Geometry check sheet. Reference: the model listing, model coordinates, mm. A direction names the side the tool comes from. Coordinates: 2 decimals unless noted, no trailing zeros. Write each loop counter-clockwise with the first axis right and the second up, starting at its lowest first coordinate (ties: lowest second). Pieces come first, ordered by that corner, then holes. Notation, with made-up numbers: M 53.5,47.25 L 94.5,47.25 A14 ccw 94.5,70.25 Z; hole C 22.25,20.5 d3. An arc over 180 degrees is marked long. Write each question's results on one line, items separated by ' | '.
```python
from build123d import *

# Parameters (mm, degrees)
BOSS_EXTRUDE1_DEPTH                                = 75
HOLE_SIZE_SOCKET_HEAD_CAP_SCREW_TYPE_1_D           = 4.5
HOLE_SIZE_SOCKET_HEAD_CAP_SCREW_TYPE_1_CBORE_D     = 8
HOLE_SIZE_SOCKET_HEAD_CAP_SCREW_TYPE_1_CBORE_DEPTH = 4.6
M5_TAPPED_HOLE1_D                                  = 4.2
M5_TAPPED_HOLE1_DEPTH                              = 12.4
M5_TAPPED_HOLE1_TIP                                = 1.2618073
M5_TAPPED_HOLE2_D                                  = 4.2
M5_TAPPED_HOLE2_DEPTH                              = 12.4
M5_TAPPED_HOLE2_TIP                                = 1.2618073
CHAMFER1_SIZE                                      = 1
DOWEL_HOLE1_D                                      = 5
DOWEL_HOLE1_DEPTH                                  = 7.5
DOWEL_HOLE1_TIP                                    = 1.502151548


with BuildPart() as part:
    # Sketch1 → Boss-Extrude1 (new, symmetric)
    with BuildSketch(Plane.XY):
        Polygon((0, 0), (0, 22), (-38, 22), (-38, 2), (-2, 2), (-2, 0), align=None)
    extrude(amount=BOSS_EXTRUDE1_DEPTH, both=True)

    # Hole size (socket head cap screw type)1 (through all)
    with Locations(Plane(origin=(0, 22, 0), x_dir=(1, 0, 0), z_dir=(0, 1, 0))):
        with Locations((-32, -68.3), (-32, 68.3), (-6, 42.3), (-32, 42.3), (-6, 68.3), (-6, -68.3), (-6, -42.3), (-32, -42.3)):
            CounterBoreHole(HOLE_SIZE_SOCKET_HEAD_CAP_SCREW_TYPE_1_D / 2, HOLE_SIZE_SOCKET_HEAD_CAP_SCREW_TYPE_1_CBORE_D / 2, HOLE_SIZE_SOCKET_HEAD_CAP_SCREW_TYPE_1_CBORE_DEPTH)

    # M5 Tapped Hole1
    with Locations(Plane(origin=(0, 0, 0), x_dir=(0, 0, -1), z_dir=(1, 0, 0))):
        with Locations((0, 12), (-25, 12), (25, 12)):
            Hole(M5_TAPPED_HOLE1_D / 2, depth=M5_TAPPED_HOLE1_DEPTH)
            with Locations((0, 0, -(M5_TAPPED_HOLE1_DEPTH + M5_TAPPED_HOLE1_TIP / 2))):  # 118° drill point
                Cone(0, M5_TAPPED_HOLE1_D / 2, M5_TAPPED_HOLE1_TIP, mode=Mode.SUBTRACT)

    # M5 Tapped Hole2
    with Locations(Plane(origin=(0, 22, 0), x_dir=(1, 0, 0), z_dir=(0, 1, 0))):
        with Locations((-19, -16.3), (-19, 68.3), (-19, 42.3), (-19, -42.3), (-19, -68.3), (-19, 16.3)):
            Hole(M5_TAPPED_HOLE2_D / 2, depth=M5_TAPPED_HOLE2_DEPTH)
            with Locations((0, 0, -(M5_TAPPED_HOLE2_DEPTH + M5_TAPPED_HOLE2_TIP / 2))):  # 118° drill point
                Cone(0, M5_TAPPED_HOLE2_D / 2, M5_TAPPED_HOLE2_TIP, mode=Mode.SUBTRACT)

    # Chamfer1
    chamfer1_edges = [part.edges().sort_by_distance(p)[0] for p in [
        (-38, 12, 75),
        (-38, 12, -75),
        (0, 11, -75),
        (0, 11, 75),
    ]]
    chamfer(chamfer1_edges, length=CHAMFER1_SIZE)

    # Dowel Hole1
    with Locations(Plane(origin=(0, 22, 0), x_dir=(1, 0, 0), z_dir=(0, 1, 0))):
        with Locations((-19, 0)):
            Hole(DOWEL_HOLE1_D / 2, depth=DOWEL_HOLE1_DEPTH)
            with Locations((0, 0, -(DOWEL_HOLE1_DEPTH + DOWEL_HOLE1_TIP / 2))):  # 118° drill point
                Cone(0, DOWEL_HOLE1_D / 2, DOWEL_HOLE1_TIP, mode=Mode.SUBTRACT)


solid = part.part
```
Q1. Sectioned sample at A-A on x = -6. Give the number of separate pieces and of enclosed holes in the cut face, and give its area (3 significant figures).
Geometry check:
separate pieces: 5 | enclosed holes: 3 | area: 2,530 mm2
Q2. Depth check by flat-ended pin: P1, Ø5, axis at x = -6, z = -42.3, coming from the +Y side; P2, Ø6, axis at x = -6, z = 68.3, coming from the -Y side. Enter the tip coordinate at first touch or a pass-through.
Geometry check:
P1: stops at y = 17.4 | P2: stops at y = 2
Q3. Access from +Z, -Z, +X, -X, +Y, -Y to the whole of each face (thin tool, end or side, straight path). Record for faces 4 (the flat face through (-38, 12, 1)), 5 (the cylindrical face through (-6.287, 14.082, -0.273)), 6 (the cylindrical face through (-32.521, 19.732, -46.266)).
Geometry check:
face 4: +Z, -Z, -X, +Y, -Y | face 5: +X | face 6: +Y
Q4. Sectioned sample at B-B on z = -34. Record the cut outline in (x, y), and give its area (3 significant figures).
Geometry check:
outline: M -38,2 L -2,2 L -2,0 L 0,0 L 0,22 L -38,22 Z | area: 764 mm2
Q5. Mould release check, pull along Z, two halves, no side actions. Record for faces 1 (the cylindrical face through (-33.038, 9.592, -40.304)), 2 (the flat face through (-19, 14, 75)), 3 (the flat face through (-20, 2, 1)): pulls with the +Z half, pulls with the -Z half, needs draft (parallel to the pull), parting line crosses it, or undercut.
Geometry check:
face 1: undercut | face 2: pulls with the +Z half | face 3: needs draft
Q6. Scan lines: probe 1 along Z at (x, y) = (-6, 18.5); probe 2 along X at (y, z) = (4.25, 42); probe 3 along X at (y, z) = (17.5, 68.3). Record each from-to range of solid material in increasing order.
Geometry check:
probe 1: z = -75 to -72.3, -64.3 to -46.3, -38.3 to 38.3, 46.3 to 64.3, 72.3 to 75 | probe 2: x = -38 to -34.23, -29.77 to -8.23, -3.77 to 0 | probe 3: x = -38 to -36, -28 to -21.1, -16.9 to -10, -2 to 0
